Source: three-view drawing plus pictorial views. Frame: mm from the lowest corner of the part. A direction names the side the tool comes from. Coordinates: 2 decimals unless noted, no trailing zeros. Order: outer loops, then holes, each group sorted by start corner. A loop starts at its lowest first (then second) coordinate and runs counter-clockwise, first axis right, second up. Notation, with made-up numbers: M 1,39.5 L 12,39.5 A16 cw 12,58.5 Z; hole C 9.5,51.25 d4. An arc over 180 degrees is marked long. One line per question, with ' | ' between items.
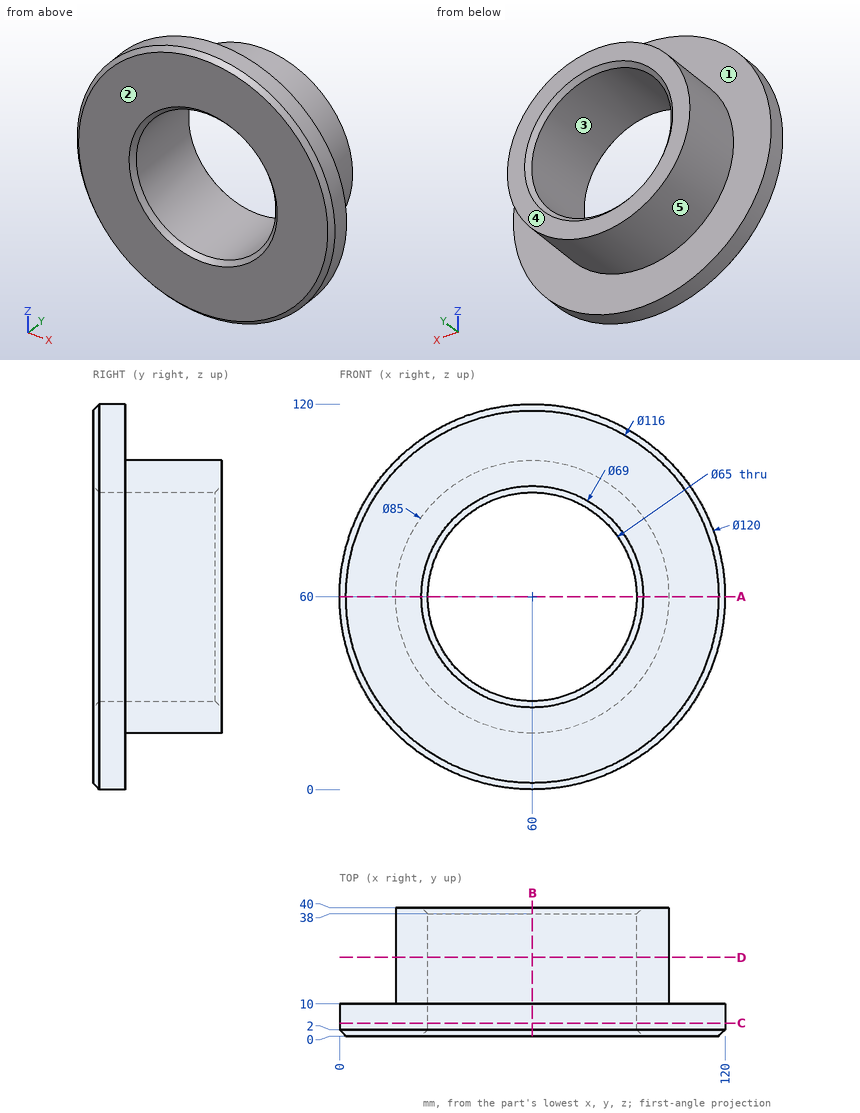
1. Section A-A, the plane z = 60. Output: boundary loops of the cut face in (x, y), and give its area (3 significant figures).
Response values:
outline: M 0,2 L 2,0 L 25.5,0 L 27.5,2 L 27.5,38 L 25.5,40 L 17.5,40 L 17.5,10 L 0,10 Z; M 92.5,2 L 94.5,0 L 118,0 L 120,2 L 120,10 L 102.5,10 L 102.5,40 L 94.5,40 L 92.5,38 Z | area: 1,140 mm^2
2. Section D-D, the plane y = 24.5. Output: boundary loops of the cut face in (x, z), and give its area (3 significant figures).
Response values:
outline: C 60,60 d85; hole C 60,60 d65 | area: 2,360 mm^2
3. Section C-C, the plane y = 4. Output: boundary loops of the cut face in (x, z), and give its area (3 significant figures).
Response values:
outline: C 60,60 d120; hole C 60,60 d65 | area: 7,990 mm^2
4. Access query for the marked faces 1 and 2. Directions: +Z, -Z, +X, -X, +Y, -Y. A direction counts if a zero-diameter tool reaches every point of the face in a straight line with its end or side. Return the directions, or none.
Response values:
face 1: +Y | face 2: +Z, -Z, +X, -X, -Y
5. Draft query along Z for the marked faces 3, 4 and 5. Return one class per face: pulls with the +Z half, pulls with the -Z half, needs draft (parallel to the pull), parting line crosses it, or undercut.
Response values:
face 3: undercut | face 4: needs draft | face 5: parting line crosses it
6. Pin query (flat end, axial travel): P1, Ø6, axis at y = 5, z = 56.5, coming from the -X side; P2, Ø3, axis at x = 34.5, z = 16.5, coming from the +Y side; P3, Ø8, axis at x = 91.5, y = 25, coming from the -Z side. Return the tip coordinate at first contact, or that it passes through.
Response values:
P1: stops at x = 0 | P2: stops at y = 10 | P3: stops at z = 27.6
7. Material intervals for line 1 (X direction, y = 16, z = 60); line 2 (Y direction, x = 51, z = 16.5); line 3 (X direction, y = 11, z = 68.5), sorted ascending. Write a range as [from, to].
Response values:
line 1: x = [17.5, 27.5], [92.5, 102.5] | line 2: y = [0, 10] | line 3: x = [18.36, 28.63], [91.37, 101.64]
8. Section B-B, the plane x = 60. Output: boundary loops of the cut face in (y, z).
Response values:
outline: M 0,2 L 2,0 L 10,0 L 10,17.5 L 40,17.5 L 40,25.5 L 38,27.5 L 2,27.5 L 0,25.5 Z; M 0,94.5 L 2,92.5 L 38,92.5 L 40,94.5 L 40,102.5 L 10,102.5 L 10,120 L 2,120 L 0,118 Z
